Job drawing, mm, ordinate dimensions from the low corner. One solid piece. A direction names the side the tool comes from. Give positions to 0.01 mm unless a question says otherwise; leave off trailing zeros. Loops run counter-clockwise (first coordinate to the right, second up) from the corner with the lowest first, then second, coordinate; pieces in that order, holes last. Notation, with made-up numbers: (11, 81.5) -> (50, 81.5) arc R14 ccw to (50, 100.5) -> close; hole circle Ø7 at (57.5, -27). An arc over 180 degrees is marked (long way). Answer as a JSON object with one key per item and string values. Group by question number.
Q1. Band-saw the part on A-A, the plane z = 3. Write the cut outline in (x, y), plus the area to 3 significant figures.
Q2. Band-saw the part on D-D, the plane y = 2.75. Write the cut outline in (x, z), plus the area to 3 significant figures.
Q3. Tool access for the marked faces 4 and 5: list every direction of +Z, -Z, +X, -X, +Y, -Y with a clear straight run to the whole face (end or side of a thin tool).
Q4. Band-saw the part on B-B, the plane y = 5. Write the cut outline in (x, z).
Q5. Drop flat-ended pins along their axis: pin 1 (2.5 mm diameter, centred on y = 5, z = 3, fed in from +X); pin 2 (2 mm diameter, centred on y = 8, z = 4, fed in from +X); pin 3 (1.8 mm diameter, centred on x = 6.5, z = 1.5, fed in from +Y). Give the stop position or say it passes through.
Q6. Two-plate mould, pull along Y, no slides. Class the marked faces 1, 2 and 3: pulls with the +Y half, pulls with the -Y half, needs draft (parallel to the pull), parting line crosses it, or undercut.
Q7. Wall check: probe 1 along Z at (x, y) = (5, 1.65); probe 2 along X at (y, z) = (7.75, 3.75); probe 3 along X at (y, z) = (2.5, 3.75). Give the ranges that are in metal, low to high. Write a range as from..to.
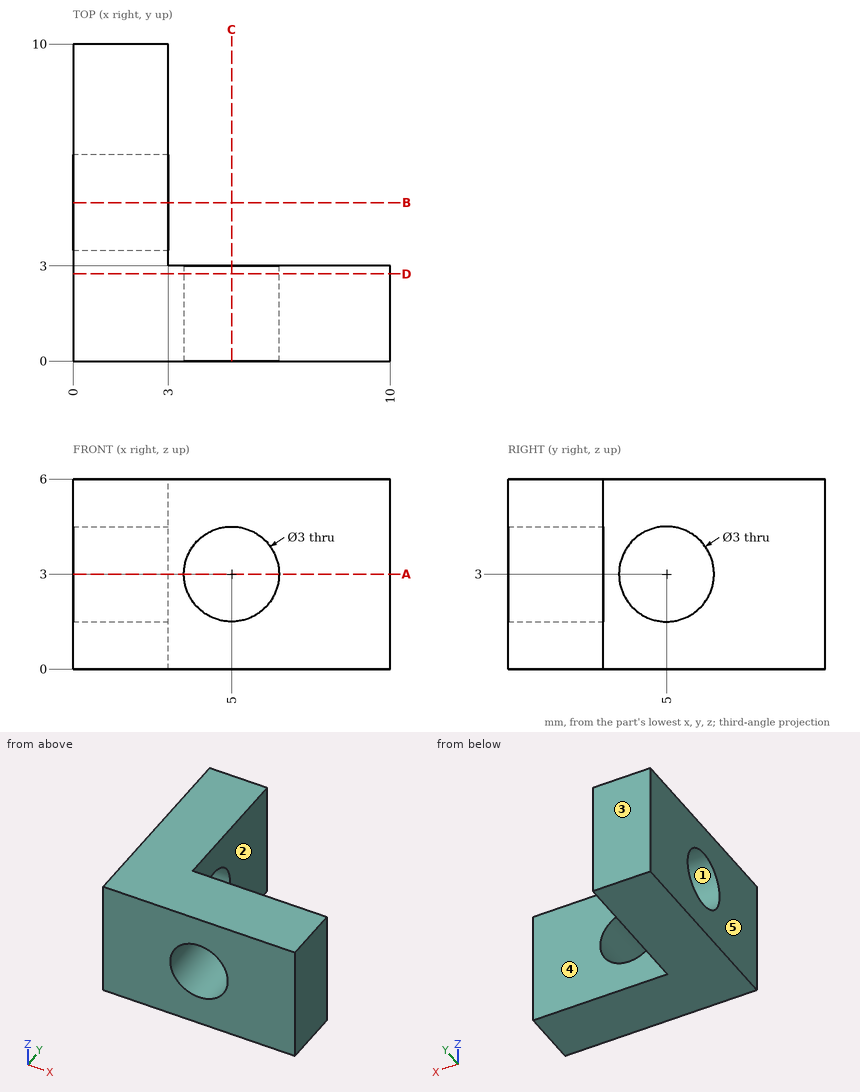
Worked answers:
{
 "1": {"outline": "(0, 0) -> (3.5, 0) -> (3.5, 3) -> (3, 3) -> (3, 3.5) -> (0, 3.5) -> close; (0, 6.5) -> (3, 6.5) -> (3, 10) -> (0, 10) -> close; (6.5, 0) -> (10, 0) -> (10, 3) -> (6.5, 3) -> close", "area": "33.0 mm2"},
 "2": {"outline": "(0, 0) -> (10, 0) -> (10, 6) -> (0, 6) -> close; hole circle Ø3 at (5, 3)", "area": "52.9 mm2"},
 "3": {"face 4": "+Z, -Z, +X, +Y", "face 5": "+Z, -Z, -X, +Y, -Y"},
 "4": {"outline": "(0, 0) -> (3, 0) -> (3, 1.5) -> (0, 1.5) -> close; (0, 4.5) -> (3, 4.5) -> (3, 6) -> (0, 6) -> close"},
 "5": {"pin 1": "through", "pin 2": "x = 3", "pin 3": "y = 3"},
 "6": {"face 1": "undercut", "face 2": "needs draft", "face 3": "pulls with the +Y half"},
 "7": {"probe 1": "0..1.5, 4.5..6", "probe 2": "0..3", "probe 3": "0..3.7, 6.3..10"}
}
